Job drawing, mm, ordinate dimensions from the low corner. One solid piece. Round coordinates to 2 decimals unless told otherwise and drop trailing zeros. Loops run counter-clockwise (first coordinate to the right, second up) from the corner with the lowest first, then second, coordinate; pieces in that order, holes last. Notation, with made-up numbers: M -31.5,70 L -17.5,70 A29 ccw -17.5,92 Z; hole C 7,23.5 d2. An arc over 180 degrees is marked long. Use one line per item in the form item = value. Start each with the question number.
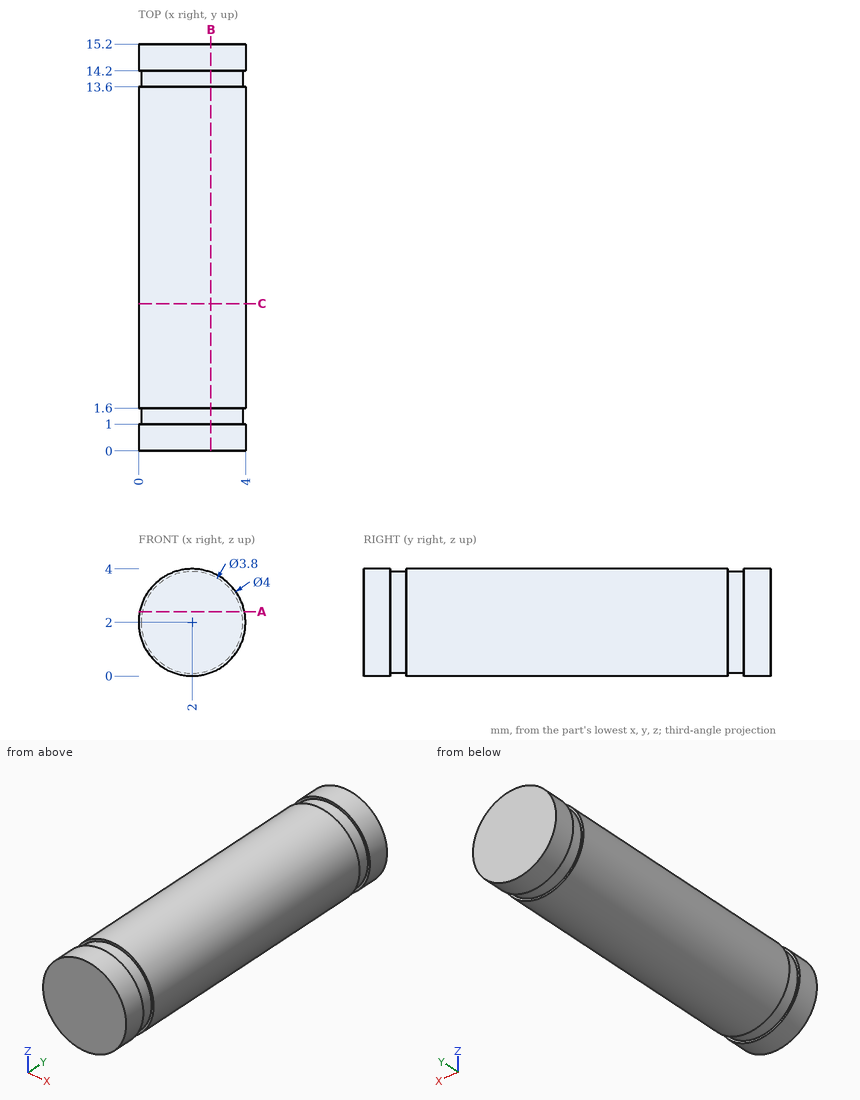
Q1. Saw through at A-A (z = 2.4). Give the cut face in (x, y), and give its area (3 significant figures).
Q2. Saw through at B-B (x = 2.7). Give the cut face in (y, z).
Q3. Wall check: probe 1 along X at (y, z) = (13.75, 2.05); probe 2 along X at (y, z) = (5.25, 2.1); probe 3 along Z at (x, y) = (1.1, 8.25). Give the ranges that are in metal, low to high.
Q4. Saw through at C-C (y = 5.5). Give the cut face in (x, z).
Filled in:
q1.outline = M 0.04,0 L 3.96,0 L 3.96,1 L 3.86,1 L 3.86,1.6 L 3.96,1.6 L 3.96,13.6 L 3.86,13.6 L 3.86,14.2 L 3.96,14.2 L 3.96,15.2 L 0.04,15.2 L 0.04,14.2 L 0.14,14.2 L 0.14,13.6 L 0.04,13.6 L 0.04,1.6 L 0.14,1.6 L 0.14,1 L 0.04,1 Z
q1.area = 59.3 mm²
q2.outline = M 0,0.13 L 1,0.13 L 1,0.23 L 1.6,0.23 L 1.6,0.13 L 13.6,0.13 L 13.6,0.23 L 14.2,0.23 L 14.2,0.13 L 15.2,0.13 L 15.2,3.87 L 14.2,3.87 L 14.2,3.77 L 13.6,3.77 L 13.6,3.87 L 1.6,3.87 L 1.6,3.77 L 1,3.77 L 1,3.87 L 0,3.87 Z
q3.probe_1 = 0.1 to 3.9
q3.probe_2 = 0 to 4
q3.probe_3 = 0.21 to 3.79
q4.outline = C 2,2 d4
